Model file for the job. Use its own axes, mm. Give positions to 0.01 mm unless a question says otherwise; leave off trailing zeros. Loops run counter-clockwise (first coordinate to the right, second up) from the corner with the lowest first, then second, coordinate; pieces in that order, holes last. Notation, with made-up numbers: M -22,13 L -15,13 A14 cw -15,27 Z; hole C -10,-13 d1. An arc over 180 degrees is marked long. Use CSV: the item, a comma, the result in double quotes. Start each with the question number.
(1) Slice it at D-D on x = 745. List the corners of the cut face in (y, z).
(2) Slice it at C-C on x = 990.5. List the corners of the cut face in (y, z).
(3) Wall check: line 1 along Z through (x, y) = (58, 143.5); line 2 along Y through (x, z) = (754, 1056); line 3 along Z through (x, y) = (204, 439). Give the ranges that are in metal, low to high. Write a range as from..to.
(4) Slice it at A-A on z = 640. List the corners of the cut face in (x, y), and give its area (3 significant figures).
(5) Slice it at B-B on y = 179. List the corners of the cut face in (x, z).
```python
from build123d import *

# Parameters (mm, degrees)
SKETCH1_W           = 1395
SKETCH1_H           = 1395
SKETCH1_W_2         = 1195
SKETCH1_H_2         = 235
BOSS_EXTRUDE1_DEPTH = 100
SKETCH2_W           = 100
SKETCH2_H           = 100
BOSS_EXTRUDE2_DEPTH = 1350
SKETCH3_W           = 100
SKETCH3_H           = 100
BOSS_EXTRUDE3_DEPTH = 1200
SKETCH4_W           = 100
SKETCH4_H           = 100
BOSS_EXTRUDE4_DEPTH = 1200


with BuildPart() as part:
    # Sketch1 → Boss-Extrude1 (new body)
    with BuildSketch(Plane.XY):
        with Locations((697.5, 697.5)):
            Rectangle(SKETCH1_W, SKETCH1_H)
        with Locations((697.5, 217.5)):
            Rectangle(SKETCH1_W_2, SKETCH1_H_2, mode=Mode.SUBTRACT)
        Polygon((100, 1295), (628.279155036, 1295), (130, 435), (100, 435), align=None, mode=Mode.SUBTRACT)
        Polygon((766.720844964, 1295), (1265, 435), (1295, 435), (1295, 1295), align=None, mode=Mode.SUBTRACT)
        Polygon((697.5, 1215), (1149.42760573, 435), (245.57239427, 435), align=None, mode=Mode.SUBTRACT)
    extrude(amount=BOSS_EXTRUDE1_DEPTH)

    # Sketch2 → Boss-Extrude2 (add)
    with BuildSketch(Plane.XY.offset(100)):
        with Locations((50, 1345)):
            Rectangle(SKETCH2_W, SKETCH2_H)
        with Locations((1345, 1345)):
            Rectangle(SKETCH2_W, SKETCH2_H)
        with Locations((50, 50)):
            Rectangle(SKETCH2_W, SKETCH2_H)
        with Locations((1345, 50)):
            Rectangle(SKETCH2_W, SKETCH2_H)
    extrude(amount=BOSS_EXTRUDE2_DEPTH)

    # Sketch3 → Boss-Extrude3 (add)
    with BuildSketch(Plane(origin=(100, 0, 0), x_dir=(0, 0, -1), z_dir=(1, 0, 0))):
        with Locations((-1100, 50)):
            Rectangle(SKETCH3_W, SKETCH3_H)
        with Locations((-1100, 1345)):
            Rectangle(SKETCH3_W, SKETCH3_H)
    extrude(amount=BOSS_EXTRUDE3_DEPTH)

    # Sketch4 → Boss-Extrude4 (add)
    with BuildSketch(Plane(origin=(0, 100, 0), x_dir=(1, 0, 0), z_dir=(0, 1, 0))):
        with Locations((50, -1100)):
            Rectangle(SKETCH4_W, SKETCH4_H)
        with Locations((1345, -1100)):
            Rectangle(SKETCH4_W, SKETCH4_H)
    extrude(amount=BOSS_EXTRUDE4_DEPTH)


solid = part.part
```
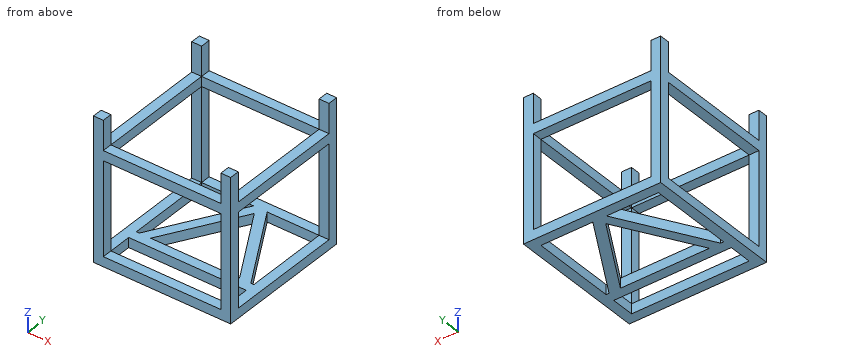
Reply:
1,outline,"M 0,0 L 100,0 L 100,100 L 0,100 Z; M 0,1050 L 100,1050 L 100,1150 L 0,1150 Z; M 335,0 L 435,0 L 435,100 L 335,100 Z; M 1133.02,0 L 1395,0 L 1395,100 L 1133.02,100 Z; M 1295,1050 L 1395,1050 L 1395,1150 L 1295,1150 Z"
2,outline,"M 0,0 L 100,0 L 100,100 L 0,100 Z; M 0,1050 L 100,1050 L 100,1150 L 0,1150 Z; M 335,0 L 435,0 L 435,100 L 335,100 Z; M 709.3,0 L 908.77,0 L 908.77,100 L 709.3,100 Z; M 1295,0 L 1395,0 L 1395,100 L 1295,100 Z; M 1295,1050 L 1395,1050 L 1395,1150 L 1295,1150 Z"
3,line 1,"z = 0..100, 1050..1150"
3,line 2,"y = 0..100, 1295..1395"
3,line 3,"z = 0..100"
4,outline,"M 0,0 L 100,0 L 100,100 L 0,100 Z; M 0,1295 L 100,1295 L 100,1395 L 0,1395 Z; M 1295,0 L 1395,0 L 1395,100 L 1295,100 Z; M 1295,1295 L 1395,1295 L 1395,1395 L 1295,1395 Z"
4,area,"40,000 mm^2"
5,outline,"M 0,0 L 100,0 L 100,100 L 0,100 Z; M 0,1050 L 100,1050 L 100,1150 L 0,1150 Z; M 1295,0 L 1395,0 L 1395,100 L 1295,100 Z; M 1295,1050 L 1395,1050 L 1395,1150 L 1295,1150 Z"
